```python
from build123d import *

# Parameters (mm, degrees)
SKETCH1_W                  = 8
SKETCH1_H                  = 3.5
BOSS_EXTRUDE1_DEPTH        = 1.5
SKETCH2_R                  = 1.25
CUT_EXTRUDE1_DEPTH         = 2
CHAMFER1_SIZE              = 0.5
F_1_0_1_DIAMETER_HOLE1_D   = 1
F_2_5_2_5_DIAMETER_HOLE1_D = 2.5


with BuildPart() as part:
    # Sketch1 → Boss-Extrude1 (new, symmetric)
    with BuildSketch(Plane(origin=(0, 0, 0), x_dir=(1, 0, 0), z_dir=(0, 1, 0))):
        Rectangle(SKETCH1_W, SKETCH1_H)
    extrude(amount=BOSS_EXTRUDE1_DEPTH, both=True)

    # Sketch2 → Cut-Extrude1 (cut)
    with BuildSketch(Plane(origin=(0, 1.5, 0), x_dir=(1, 0, 0), z_dir=(0, 1, 0))):
        with Locations(Location((-2, 0, 0), (0, 0, 270))):
            Circle(SKETCH2_R)
    extrude(amount=-CUT_EXTRUDE1_DEPTH, mode=Mode.SUBTRACT)

    # Chamfer1
    chamfer1_edges = [part.edges().sort_by_distance(p)[0] for p in [
        (4, 0, 1.75),
        (-4, 0, 1.75),
        (-4, 0, -1.75),
        (4, 0, -1.75),
    ]]
    chamfer(chamfer1_edges, length=CHAMFER1_SIZE)

    # Ø1.0 (1) Diameter Hole1 (through all)
    with Locations(Plane(origin=(0, -1.5, 0), x_dir=(-1, 0, 0), z_dir=(0, -1, 0))):
        with Locations((2, 0)):
            Hole(F_1_0_1_DIAMETER_HOLE1_D / 2)

    # Ø2.5 (2.5) Diameter Hole1 (through all)
    with Locations(Plane(origin=(0, -1.5, 0), x_dir=(-1, 0, 0), z_dir=(0, -1, 0))):
        with Locations((-2, 0)):
            Hole(F_2_5_2_5_DIAMETER_HOLE1_D / 2)


solid = part.part
```
For this review, take the finished solid that the model builds, in its own axes (mm). A direction names the side the tool comes from. Coordinates: 2 decimals unless noted, no trailing zeros. Write each loop counter-clockwise with the first axis right and the second up, starting at its lowest first coordinate (ties: lowest second). Pieces come first, ordered by that corner, then holes. Notation, with made-up numbers: (6.25, 42) - (64.25, 42) arc R21 cw to (64.25, 61) - close; hole circle Ø1 at (-18.5, 54). An arc over 180 degrees is marked (long way). Put each result on its own line as item: value.
1. Add section A-A, the plane x = 2. Give the boundary of the cut face in (y, z).
Values found:
outline: (-1.5, -1.75) - (1.5, -1.75) - (1.5, -1.25) - (-1.5, -1.25) - close; (-1.5, 1.25) - (1.5, 1.25) - (1.5, 1.75) - (-1.5, 1.75) - close
2. Add section B-B, the plane z = 0. Give the boundary of the cut face in (x, y).
Values found:
outline: (-4, -1.5) - (-2.5, -1.5) - (-2.5, -0.5) - (-3.25, -0.5) - (-3.25, 1.5) - (-4, 1.5) - close; (-1.5, -1.5) - (0.75, -1.5) - (0.75, 1.5) - (-0.75, 1.5) - (-0.75, -0.5) - (-1.5, -0.5) - close; (3.25, -1.5) - (4, -1.5) - (4, 1.5) - (3.25, 1.5) - close
3. Machinability: for faces 1 (the flat face through (0, 1.5, 0)), 2 (the cylindrical face through (-0.76, 0.51, -0.16)), which of the approach directions +Z, -Z, +X, -X, +Y, -Y give a long, thin tool a straight path to every point of the face, cutting with its end or side? Answer none if there is none.
Values found:
face 1: +Z, -Z, +X, -X, +Y
face 2: +Y
4. For pin 1 (1.2 mm diameter, centred on x = -2, z = 0.5, fed in from +Y), flat-tipped, find the tip position at first contact; note if it passes through.
Values found:
pin 1: y = -0.5
5. Add section D-D, the plane z = -0.7. Give the boundary of the cut face in (x, y), then the cut area to 3 significant figures.
Values found:
outline: (-4, -1.5) - (0.96, -1.5) - (0.96, 1.5) - (-0.96, 1.5) - (-0.96, -0.5) - (-3.04, -0.5) - (-3.04, 1.5) - (-4, 1.5) - close; (3.04, -1.5) - (4, -1.5) - (4, 1.5) - (3.04, 1.5) - close
area: 13.6 mm²
6. Wall thickness on probe 1 along Z at (x, y) = (2, 0.6); probe 2 along Z at (x, y) = (-2, -1.3); probe 3 along X at (y, z) = (0.7, 0.9): over which ranges is each line inside the solid? List them lowest first.
Values found:
probe 1: -1.75 to -1.25, 1.25 to 1.75
probe 2: -1.75 to -0.5, 0.5 to 1.75
probe 3: -4 to -2.87, -1.13 to 1.13, 2.87 to 4
7. Mouldability with a two-part tool opening along X and no side actions: class faces 3 (the flat face through (0, 0, -1.75)), 4 (the flat face through (-4, 0, 0)), 5 (the cylindrical face through (-2.4, -1, 0.3)) as released by +X, released by -X, zero draft, split by the parting line, or undercut.
Values found:
face 3: zero draft
face 4: released by -X
face 5: undercut
8. Add section C-C, the plane y = 0.35. Give the boundary of the cut face in (x, z).
Values found:
outline: (-4, -1.25) - (-3.5, -1.75) - (3.5, -1.75) - (4, -1.25) - (4, 1.25) - (3.5, 1.75) - (-3.5, 1.75) - (-4, 1.25) - close; hole circle Ø2.5 at (-2, 0); hole circle Ø2.5 at (2, 0)
